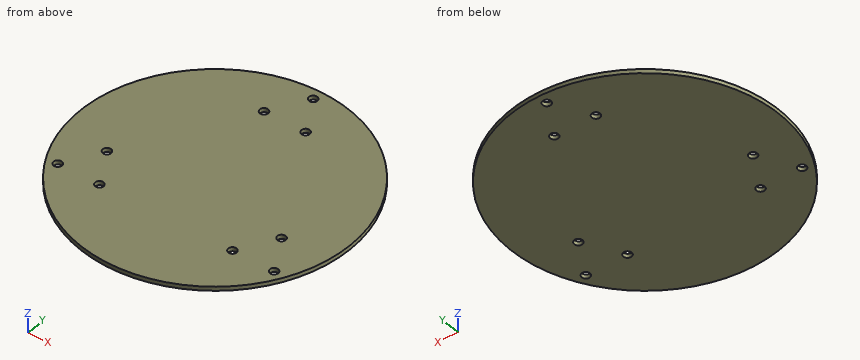
```python
from build123d import *

# Parameters (mm, degrees)
SKETCH1_R           = 65
BOSS_EXTRUDE1_DEPTH = 2
SKETCH3_R           = 2
CUT_EXTRUDE1_DEPTH  = 92.945636112


with BuildPart() as part:
    # Sketch1 → Boss-Extrude1 (new body)
    with BuildSketch(Plane.XY):
        Circle(SKETCH1_R)
    extrude(amount=BOSS_EXTRUDE1_DEPTH)

    # Sketch3 → Cut-Extrude1 (cut, through all)
    with BuildSketch(Plane.XY.offset(2)):
        with Locations((0, 60)):
            Circle(SKETCH3_R)
        with Locations((10, 42.679491924)):
            Circle(SKETCH3_R)
        with Locations((-10, 42.679491924)):
            Circle(SKETCH3_R)
        with Locations((31.961524227, -30)):
            Circle(SKETCH3_R)
        with Locations((41.961524227, -12.679491924)):
            Circle(SKETCH3_R)
        with Locations((51.961524227, -30)):
            Circle(SKETCH3_R)
        with Locations((-41.961524227, -12.679491924)):
            Circle(SKETCH3_R)
        with Locations((-31.961524227, -30)):
            Circle(SKETCH3_R)
        with Locations((-51.961524227, -30)):
            Circle(SKETCH3_R)
    extrude(amount=-CUT_EXTRUDE1_DEPTH, mode=Mode.SUBTRACT)


solid = part.part
```
Verification items for the finished model (mm, model axes). Round coordinates to 2 decimals unless told otherwise and drop trailing zeros. Order: outer loops, then holes, each group sorted by start corner. A loop starts at its lowest first (then second) coordinate and runs counter-clockwise, first axis right, second up.
1) Material ranges on line 1 (Y direction, x = 0, z = 1.1); line 2 (Y direction, x = 10, z = 1.25); line 3 (X direction, y = -2, z = 1.85), recorded low to high.
Geometry says:
line 1: y = -65 to 58, 62 to 65
line 2: y = -64.23 to 40.68, 44.68 to 64.23
line 3: x = -64.97 to 64.97
2) Cross-section at B-B, the plane y = 60. Record the cut outline in (x, z).
Geometry says:
outline: (-25, 0) - (-2, 0) - (-2, 2) - (-25, 2) - close; (2, 0) - (25, 0) - (25, 2) - (2, 2) - close
3) Cross-section at A-A, the plane x = 0. Record the cut outline in (y, z), plus the area to 3 significant figures.
Geometry says:
outline: (-65, 0) - (58, 0) - (58, 2) - (-65, 2) - close; (62, 0) - (65, 0) - (65, 2) - (62, 2) - close
area: 252 mm2
4) Cross-section at D-D, the plane z = 0.4. Give the number of separate pieces and of enclosed holes in the cut face, plus the area to 3 significant figures.
Geometry says:
separate pieces: 1
enclosed holes: 9
area: 13,200 mm2
5) Depth check by flat-ended pin: pin 1 (3.5 mm diameter, centred on x = -41.96, y = -12.68, fed in from +Z); pin 2 (1 mm diameter, centred on y = 14, z = 1, fed in from +X). Enter the tip coordinate at first touch or a pass-through.
Geometry says:
pin 1: passes through
pin 2: stops at x = 63.58
6) Cross-section at C-C, the plane y = -30. Record the cut outline in (x, z).
Geometry says:
outline: (-57.66, 0) - (-53.96, 0) - (-53.96, 2) - (-57.66, 2) - close; (-49.96, 0) - (-33.96, 0) - (-33.96, 2) - (-49.96, 2) - close; (-29.96, 0) - (29.96, 0) - (29.96, 2) - (-29.96, 2) - close; (33.96, 0) - (49.96, 0) - (49.96, 2) - (33.96, 2) - close; (53.96, 0) - (57.66, 0) - (57.66, 2) - (53.96, 2) - close
